Model file for the job. Use its own axes, mm. Round coordinates to 2 decimals unless told otherwise and drop trailing zeros. Loops run counter-clockwise (first coordinate to the right, second up) from the corner with the lowest first, then second, coordinate; pieces in that order, holes last. Notation, with made-up numbers: M -37,-4.75 L -23,-4.75 A20 cw -23,11.25 Z; hole C 33,-40 d4. An arc over 180 degrees is marked long. Answer in a Markdown table with one row per item.
from build123d import *

# Parameters (mm, degrees)
SKETCH1_W           = 230
SKETCH1_H           = 166
SKETCH1_W_2         = 210
SKETCH1_H_2         = 146
BOSS_EXTRUDE1_DEPTH = 5
FILLET1_R           = 5
FILLET2_R           = 15


with BuildPart() as part:
    # Sketch1 → Boss-Extrude1 (new body)
    with BuildSketch(Plane.XY):
        Rectangle(SKETCH1_W, SKETCH1_H)
        Rectangle(SKETCH1_W_2, SKETCH1_H_2, mode=Mode.SUBTRACT)
    extrude(amount=BOSS_EXTRUDE1_DEPTH)

    # Fillet1
    fillet1_edges = [part.edges().sort_by_distance(p)[0] for p in [
        (-105, 73, 2.5),
        (-105, -73, 2.5),
        (105, -73, 2.5),
        (105, 73, 2.5),
    ]]
    fillet(fillet1_edges, radius=FILLET1_R)

    # Fillet2
    fillet2_edges = [part.edges().sort_by_distance(p)[0] for p in [
        (-115, 83, 2.5),
        (115, 83, 2.5),
        (115, -83, 2.5),
        (-115, -83, 2.5),
    ]]
    fillet(fillet2_edges, radius=FILLET2_R)


solid = part.part
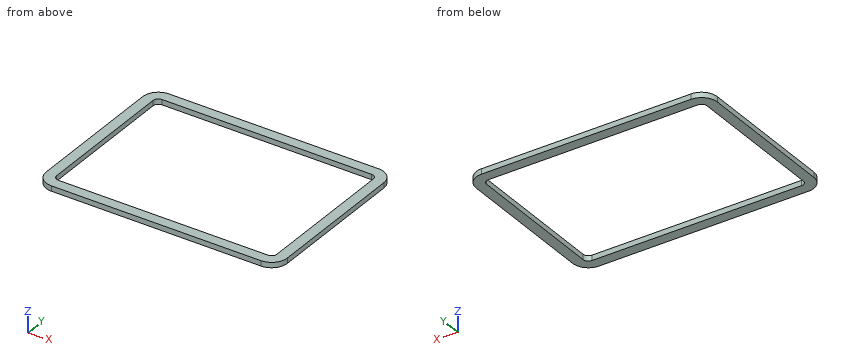
1. Saw through at B-B (x = -2). Write the cut outline in (y, z).
Verdict:
| item | result |
|---|---|
| outline | M -83,0 L -73,0 L -73,5 L -83,5 Z; M 73,0 L 83,0 L 83,5 L 73,5 Z |
2. Saw through at C-C (z = 3.2). Write the cut outline in (x, y), and give its area (3 significant figures).
Verdict:
| item | result |
|---|---|
| outline | M -115,-68 A15 ccw -100,-83 L 100,-83 A15 ccw 115,-68 L 115,68 A15 ccw 100,83 L -100,83 A15 ccw -115,68 Z; hole M -105,-68 A5 ccw -100,-73 L 100,-73 A5 ccw 105,-68 L 105,68 A5 ccw 100,73 L -100,73 A5 ccw -105,68 Z |
| area | 7,350 mm² |
3. Saw through at A-A (y = 17). Write the cut outline in (x, z).
Verdict:
| item | result |
|---|---|
| outline | M -115,0 L -105,0 L -105,5 L -115,5 Z; M 105,0 L 115,0 L 115,5 L 105,5 Z |
4. Wall check: probe 1 along Y at (x, z) = (98, 2.3); probe 2 along X at (y, z) = (61.5, 4.25); probe 3 along Y at (x, z) = (-102, 2.75). Give the ranges that are in metal, low to high.
Verdict:
| item | result |
|---|---|
| probe 1 | y = -83 to -73, 73 to 83 |
| probe 2 | x = -115 to -105, 105 to 115 |
| probe 3 | y = -82.87 to -72.58, 72.58 to 82.87 |
